Input: part model. Units: mm. Frame: model coordinates. A direction names the side the tool comes from. Round coordinates to 2 decimals unless told otherwise and drop trailing zeros. Loops run counter-clockwise (first coordinate to the right, second up) from the corner with the lowest first, then second, coordinate; pieces in that order, holes last.
(1) Cut plane B-B, the plane y = -42. Output: boundary loops of the cut face in (x, z), and give its area (3 significant figures).
(2) Access query for faces 1 (the face through (108, -1, 150)), 2 (the face through (98, 0, 73)), 3 (the face through (0, -74, 73)), 4 (the face through (98, -144, 45)), 5 (the face through (91, -146, 43)). Directions: +Z, -Z, +X, -X, +Y, -Y. A direction counts if a zero-diameter tool reaches every point of the face in a straight line with its end or side. Return the directions, or none.
(3) Draft query along X for faces 6 (the face through (198, -74, 73)), 7 (the face through (98, -72, 0)), 8 (the face through (196, -74, 75)), 9 (the face through (98, -2, 75)). Return one class per face: released by +X, released by -X, zero draft, split by the parting line, or undercut.
(4) Cut plane C-C, the plane z = 106. Output: boundary loops of the cut face in (x, y).
(5) Cut plane D-D, the plane x = 64. Output: boundary loops of the cut face in (y, z), and give its area (3 significant figures).
(6) First-contact query: pin 1 Ø2 at (x, z) = (197, 111.5) entering from -Y; pin 2 Ø1 at (y, z) = (-23.5, 131) entering from -X; pin 3 Ø1 at (x, z) = (166, 133) entering from +Y. Flat tips, straight axial feed; report the tip coordinate or a pass-through.
(7) Line query: line 1 (X direction, y = -137, z = 97.5); line 2 (Y direction, x = 25, z = 36); line 3 (Z direction, x = 135, y = -136.5). Output: solid intervals per line, ascending.
(8) Cut plane A-A, the plane z = 75. Output: boundary loops of the cut face in (x, y).
from build123d import *

# Parameters (mm, degrees)
SKETCH_1_W          = 198
SKETCH_1_H          = 146
EXTRUDE_1_DEPTH     = 150
SHELL_1_T           = -2
EXTRUDE_2_DEPTH     = 2
SKETCH_3_W          = 196
SKETCH_3_H          = 60
CUT_EXTRUDE_1_DEPTH = 2


with BuildPart() as part:
    # 草图1 → 凸台-拉伸1 (new body)
    with BuildSketch(Plane.XY):
        with Locations((99, -73)):
            Rectangle(SKETCH_1_W, SKETCH_1_H)
    extrude(amount=EXTRUDE_1_DEPTH)

    # 抽壳1
    shell_1_openings = [part.faces().sort_by_distance(p)[0] for p in [
        (99, -73, 150),
    ]]
    offset(amount=SHELL_1_T, openings=shell_1_openings, kind=Kind.INTERSECTION)

    # 草图2 → 凸台-拉伸2 (add)
    with BuildSketch(Plane.XY.offset(150)):
        Polygon((0, -146), (-20, -146), (-20, 20), (218, 20), (218, -146), (198, -146), (198, 0), (0, 0), align=None)
    extrude(amount=-EXTRUDE_2_DEPTH)

    # 草图3 → 切除-拉伸1 (cut)
    with BuildSketch(Plane.XZ.offset(146)):
        with Locations((100, 120)):
            Rectangle(SKETCH_3_W, SKETCH_3_H)
    extrude(amount=-CUT_EXTRUDE_1_DEPTH, mode=Mode.SUBTRACT)


solid = part.part
Reported:
1. outline: (-20, 148) - (0, 148) - (0, 0) - (198, 0) - (198, 148) - (218, 148) - (218, 150) - (196, 150) - (196, 2) - (2, 2) - (2, 150) - (-20, 150) - close
1. area: 1,070 mm2
2. face 1: +Z, +X, -X, +Y, -Y
2. face 2: -Z, +X, -X, +Y
2. face 3: -Z, -X, +Y, -Y
2. face 4: +Z
2. face 5: +Z, -Z, +X, -X, -Y
3. face 6: released by +X
3. face 7: zero draft
3. face 8: undercut
3. face 9: undercut
4. outline: (0, -146) - (2, -146) - (2, -2) - (196, -2) - (196, -144) - (198, -144) - (198, 0) - (0, 0) - close
5. outline: (-146, 0) - (0, 0) - (0, 148) - (20, 148) - (20, 150) - (-2, 150) - (-2, 2) - (-144, 2) - (-144, 90) - (-146, 90) - close
5. area: 804 mm2
6. pin 1: stops at y = -144
6. pin 2: stops at x = 0
6. pin 3: stops at y = 0
7. line 1: x = 0 to 2, 196 to 198
7. line 2: y = -146 to -144, -2 to 0
7. line 3: z = 0 to 2
8. outline: (0, -146) - (198, -146) - (198, 0) - (0, 0) - close; hole (2, -144) - (196, -144) - (196, -2) - (2, -2) - close
